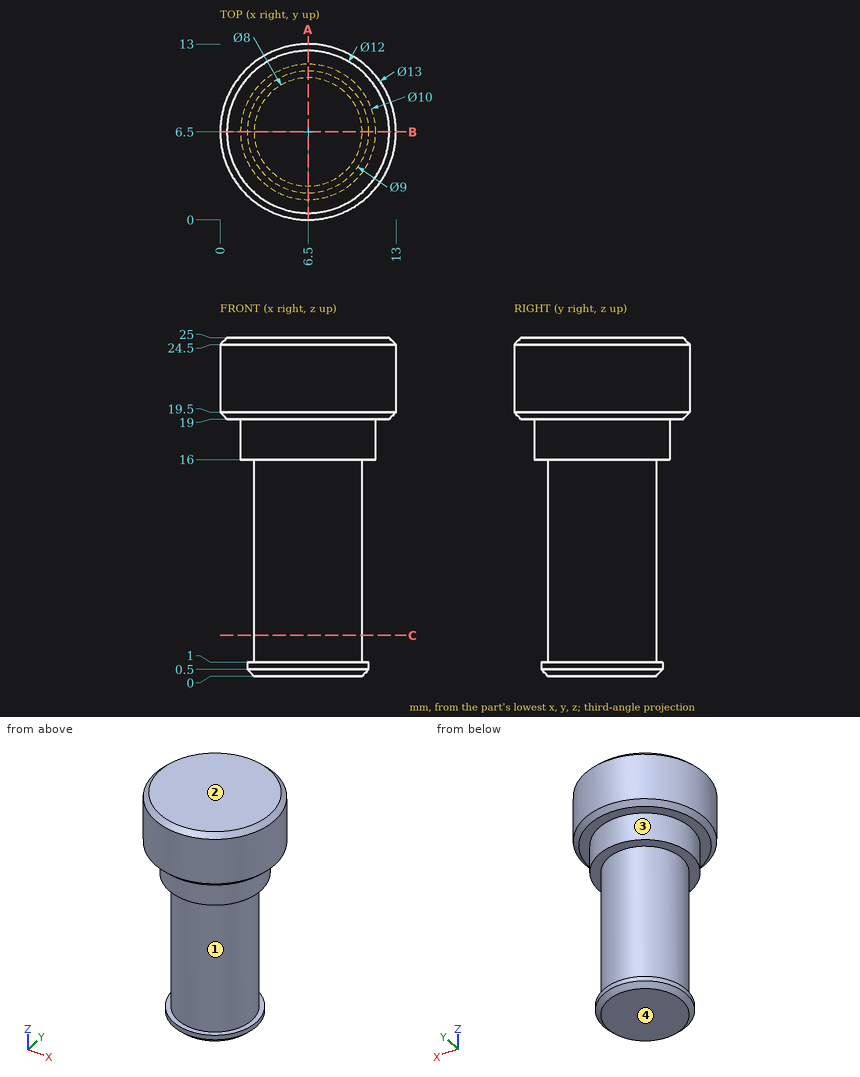
Part print with two shaded views. Sizes in mm from the minimum x, y, z corner. Round coordinates to 2 decimals unless told otherwise and drop trailing zeros. Write each loop counter-clockwise with the first axis right and the second up, starting at its lowest first coordinate (ties: lowest second). Pieces come first, ordered by that corner, then holes. Notation, with made-up numbers: (-18.75, 55.25) -> (-2.75, 55.25) arc R16 cw to (-2.75, 59.25) -> close; hole circle Ø10 at (-10, -9.5). An arc over 180 degrees is marked (long way). Use one line per item in the form item = value.
Q1. Band-saw the part on A-A, the plane x = 6.5. Write the cut outline in (y, z).
Conclusion:
outline = (0, 19.5) -> (0.5, 19) -> (1.5, 19) -> (1.5, 16) -> (2.5, 16) -> (2.5, 1) -> (2, 1) -> (2, 0.5) -> (2.5, 0) -> (10.5, 0) -> (11, 0.5) -> (11, 1) -> (10.5, 1) -> (10.5, 16) -> (11.5, 16) -> (11.5, 19) -> (12.5, 19) -> (13, 19.5) -> (13, 24.5) -> (12.5, 25) -> (0.5, 25) -> (0, 24.5) -> close
Q2. Band-saw the part on C-C, the plane z = 3. Write the cut outline in (x, y).
Conclusion:
outline = circle Ø8 at (6.5, 6.5)
Q3. Drill centre lines: L1, parallel to Z at x = 11.75, y = 5.25; L2, parallel to Y at x = 10.25, z = 23.25; L3, parallel to Y at x = 9, z = 5. Where is each one in solid material? Low to high.
Conclusion:
L1 = 19 to 25
L2 = 1.19 to 11.81
L3 = 3.38 to 9.62
Q4. Two-plate mould, pull along Z, no slides. Class the marked faces 1, 2, 3 and 4: released by +Z, released by -Z, zero draft, split by the parting line, or undercut.
Conclusion:
face_1 = undercut
face_2 = released by +Z
face_3 = zero draft
face_4 = released by -Z
Q5. Drop flat-ended pins along their axis: P1, Ø1.5, axis at y = 3.5, z = 20, coming from the +X side; P2, Ø1.5, axis at y = 3.5, z = 13, coming from the +X side. Give the stop position or say it passes through.
Conclusion:
P1 = 12.6
P2 = 9.81
